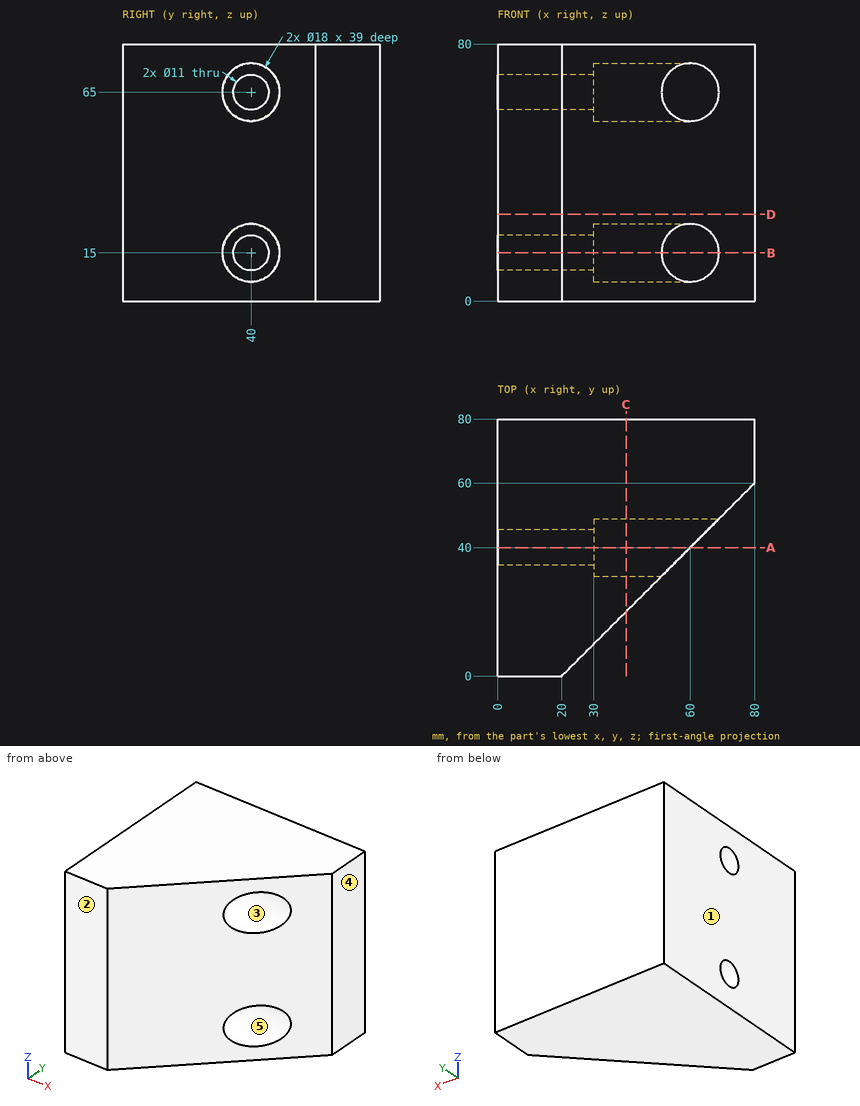
Answer from the drawing. Dimensions are ordinates in mm from the lowest x, y and z of the part. A direction names the side the tool comes from. Round coordinates to 2 decimals unless told otherwise and drop trailing zeros. Write each loop counter-clockwise with the first axis right and the second up, starting at its lowest first coordinate (ties: lowest second). Pieces come first, ordered by that corner, then holes. Notation, with made-up numbers: (85.5, 76.25) - (90.5, 76.25) arc R27 ccw to (90.5, 100.25) - close; hole circle Ø1 at (27, -19.5). An arc over 180 degrees is marked (long way). One line per item, written item: value.
Q1. Each of these flat-tipped pins is pushed along its axis until it touches: P1, Ø8, axis at y = 19, z = 60, coming from the +X side; P2, Ø1, axis at x = 70.5, z = 11.5, coming from the -Y side; P3, Ø14.5, axis at y = 41, z = 68.5, coming from the +X side. Where does it stop, or does it pass through?
The answers:
P1: stops at x = 43
P2: stops at y = 50
P3: stops at x = 68.25
Q2. Find section B-B (z = 15). Determine the outline of the cut face in (x, y), and give its area (3 significant figures).
The answers:
outline: (0, 0) - (20, 0) - (51, 31) - (30, 31) - (30, 34.5) - (0, 34.5) - close; (0, 45.5) - (30, 45.5) - (30, 49) - (69, 49) - (80, 60) - (80, 80) - (0, 80) - close
area: 3,730 mm2
Q3. Which of the six approach directions +Z, -Z, +X, -X, +Y, -Y give full straight-line access (tool end or side, diameter ignored) to the marked faces 4 and 5?
The answers:
face 4: +Z, -Z, +X, +Y, -Y
face 5: +X
Q4. Straight lines are drawn through the part: line 1 (Y direction, x = 6.5, z = 65); line 2 (Z direction, x = 55, y = 40); line 3 (Y direction, x = 49, z = 65). For each, find the intervals that lie inside material, in ascending order. Write a range as from..to.
The answers:
line 1: y = 0..34.5, 45.5..80
line 2: z = 0..6, 24..56, 74..80
line 3: y = 29..31, 49..80
Q5. For a pull along Y with two mould halves and no side action, classify the marked faces 1, 2 and 3 as pulls with the +Y half, pulls with the -Y half, needs draft (parallel to the pull), parting line crosses it, or undercut.
The answers:
face 1: needs draft
face 2: pulls with the -Y half
face 3: undercut
Q6. Find section C-C (x = 40). Determine the outline of the cut face in (y, z), and give its area (3 significant figures).
The answers:
outline: (20, 0) - (80, 0) - (80, 80) - (20, 80) - close; hole circle Ø18 at (40, 15); hole circle Ø18 at (40, 65)
area: 4,290 mm2
Q7. Find section D-D (z = 27). Determine the outline of the cut face in (x, y), and give its area (3 significant figures).
The answers:
outline: (0, 0) - (20, 0) - (80, 60) - (80, 80) - (0, 80) - close
area: 4,600 mm2
Q8. Find section A-A (y = 40). Determine the outline of the cut face in (x, z), and give its area (3 significant figures).
The answers:
outline: (0, 0) - (60, 0) - (60, 6) - (30, 6) - (30, 9.5) - (0, 9.5) - close; (0, 20.5) - (30, 20.5) - (30, 24) - (60, 24) - (60, 56) - (30, 56) - (30, 59.5) - (0, 59.5) - close; (0, 70.5) - (30, 70.5) - (30, 74) - (60, 74) - (60, 80) - (0, 80) - close
area: 3,060 mm2
